Source: CAD feature listing. Evaluate the final solid. Frame: model axes, mm. A direction names the side the tool comes from. Give positions to 0.01 mm unless a question says otherwise; leave off trailing zeros. Write each loop counter-clockwise with the first axis right and the second up, starting at its lowest first coordinate (ties: lowest second). Pieces come first, ordered by that corner, then holes. Notation, with made-up numbers: (-3, -30) - (45, -30) arc R8 cw to (45, -25) - close; hole circle Ø9 at (-32, -23.5). An arc over 180 degrees is marked (long way). One line per question, with ' | ' between items. Start each with the question number.
(1) Section D-D, the plane x = 19. Return loops of the section in (y, z).
(2) Section A-A, the plane z = 17.5. Return loops of the section in (x, y).
(3) Section B-B, the plane y = 9.8. Return loops of the section in (x, z), plus the area to 3 significant figures.
(4) Section C-C, the plane y = 0. Return loops of the section in (x, z).
(5) Pin query (flat end, axial travel): pin 1 (3.5 mm diameter, centred on x = 1, z = 25, fed in from +Y). Return the tip coordinate at first contact, or that it passes through.
(6) Draft query along X for faces 1 (the flat face through (-3.5, 3, 18)), 2 (the cylindrical face through (18.304, 7.847, 12.789)), 3 (the flat face through (3.5, 3, 18)), 4 (the flat face through (-32.7, 0, 17)). Return one class per face: +X half, -X half, draft (parallel to the pull), parting line (faces both ways), or undercut.
(7) Access query for faces 5 (the flat face through (0, -9.5, 18)), 6 (the flat face through (-18, 22.5, 17)). Directions: +Z, -Z, +X, -X, +Y, -Y. A direction counts if a zero-diameter tool reaches every point of the face in a straight line with its end or side. Return the directions, or none.
(8) Ray query, line 1 (X direction, y = 4, z = 22.5); line 2 (Y direction, x = 26.25, z = 17.5); line 3 (Z direction, x = 21, y = 9). Return the intervals inside material, ascending. Write a range as [from, to].
```python
from build123d import *

# Parameters (mm, degrees)
SKETCH_1_W          = 65.4
SKETCH_1_H          = 45
EXTRUDE_1_DEPTH     = 35
FILLET_1_R          = 10
SKETCH_2_R          = 5.1
CUT_EXTRUDE_1_DEPTH = 84
SKETCH_3_W          = 7
SKETCH_3_H          = 50
CUT_EXTRUDE_2_DEPTH = 35


with BuildPart() as part:
    # 草图1 → 凸台-拉伸1 (new body)
    with BuildSketch(Plane.XY):
        Rectangle(SKETCH_1_W, SKETCH_1_H)
    extrude(amount=EXTRUDE_1_DEPTH)

    # 圆角1
    fillet_1_edges = [part.edges().sort_by_distance(p)[0] for p in [
        (0, 22.5, 35),
        (0, 22.5, 0),
    ]]
    fillet(fillet_1_edges, radius=FILLET_1_R)

    # 草图2 → 切除-拉伸1 (cut)
    with BuildSketch(Plane(origin=(32.7, 0, 0), x_dir=(0, 0, -1), z_dir=(1, 0, 0))):
        with Locations((-17.5, 9.8)):
            Circle(SKETCH_2_R)
    extrude(amount=-CUT_EXTRUDE_1_DEPTH, mode=Mode.SUBTRACT)

    # 草图3 → 切除-拉伸2 (cut)
    with BuildSketch(Plane.XY.offset(35)):
        with Locations((0, 15.5)):
            Rectangle(SKETCH_3_W, SKETCH_3_H)
    extrude(amount=-CUT_EXTRUDE_2_DEPTH, mode=Mode.SUBTRACT)


solid = part.part
```
Check sheet entries:
1) outline: (-22.5, 0) - (12.5, 0) arc R10 ccw to (22.5, 10) - (22.5, 25) arc R10 ccw to (12.5, 35) - (-22.5, 35) - close; hole circle Ø10.2 at (9.8, 17.5)
2) outline: (-32.7, -22.5) - (32.7, -22.5) - (32.7, 4.7) - (3.5, 4.7) - (3.5, -9.5) - (-3.5, -9.5) - (-3.5, 4.7) - (-32.7, 4.7) - close; (-32.7, 14.9) - (-3.5, 14.9) - (-3.5, 22.5) - (-32.7, 22.5) - close; (3.5, 14.9) - (32.7, 14.9) - (32.7, 22.5) - (3.5, 22.5) - close
3) outline: (-32.7, 0) - (-3.5, 0) - (-3.5, 12.4) - (-32.7, 12.4) - close; (-32.7, 22.6) - (-3.5, 22.6) - (-3.5, 35) - (-32.7, 35) - close; (3.5, 0) - (32.7, 0) - (32.7, 12.4) - (3.5, 12.4) - close; (3.5, 22.6) - (32.7, 22.6) - (32.7, 35) - (3.5, 35) - close | area: 1,450 mm²
4) outline: (-32.7, 0) - (-3.5, 0) - (-3.5, 35) - (-32.7, 35) - close; (3.5, 0) - (32.7, 0) - (32.7, 35) - (3.5, 35) - close
5) pin 1: y = -9.5
6) face 1: undercut | face 2: draft | face 3: undercut | face 4: -X half
7) face 5: +Z, -Z, +Y | face 6: +Z, -Z, +X, -X, +Y
8) line 1: [-32.7, -3.5], [3.5, 32.7] | line 2: [-22.5, 4.7], [14.9, 22.5] | line 3: [0, 12.46], [22.54, 35]
